Build history of the part. All positions in model axes, mm. A direction names the side the tool comes from. Round coordinates to 2 decimals unless told otherwise and drop trailing zeros. Write each loop counter-clockwise with the first axis right and the second up, starting at its lowest first coordinate (ties: lowest second). Pieces come first, ordered by that corner, then holes.
Item 1: Band-saw the part on A-A, the plane z = 50. Write the cut outline in (x, y), then the cut area to 3 significant figures.
Item 2: Band-saw the part on C-C, the plane y = 86.5. Write the cut outline in (x, z).
Item 3: Mould opens along Z. For faces 1 (the flat face through (-1, 51, 130)), 2 (the flat face through (-7, 42, -2)), 3 (the flat face through (-75, 46, -80)), 4 (the flat face through (-75, 46, 80)) say: +Z half, -Z half, draft (parallel to the pull), parting line (faces both ways), or undercut.
Item 4: Band-saw the part on D-D, the plane x = -76. Write the cut outline in (y, z).
Item 5: Wall check: probe 1 along Z at (x, y) = (60, 15); probe 2 along Z at (x, y) = (69.5, 25.5); probe 3 along X at (y, z) = (12, -50). Give the ranges that are in metal, low to high.
Item 6: 3-axis set-ups, long thin cutter, end or side, ignore diameter. For faces 5 (the cylindrical face through (30.007, 59.704, -50.66)), 6 (the flat face through (-71, 25, 50)), 7 (the flat face through (7, 42, -2)): which of +Z, -Z, +X, -X, +Y, -Y reach the whole face in a straight line?
Item 7: Drop flat-ended pins along their axis: pin 1 Ø1.5 at (x, z) = (-45.5, 25.5) entering from +Y; pin 2 Ø18.5 at (x, y) = (-87.5, 60.5) entering from -Z; pin 3 Ø2 at (x, z) = (-32, -18) entering from -Y; pin 4 Ø2 at (x, z) = (-16.5, -0.5) entering from +Y. Give the stop position or say it passes through.
Item 8: Band-saw the part on B-B, the plane z = 3. Write the cut outline in (x, y), then the cut area to 3 significant figures.
```python
from build123d import *

# Parameters (mm, degrees)
HOUSING_BODY_DEPTH                     = 130
BOLT_START                             = 25
BOLT_POCKET_DEPTH                      = 260
BOLT_POCKET_MIRROR_RIGHT_COPY_1_DEPTH  = 260
BOLT_HOLE_SKETCH_R                     = 10
BOLT_HOLE_20_DEPTH                     = 260
BOLT_HOLE_MIRROR_RIGHT_COPY_1_SKETCH_R = 10
BOLT_HOLE_MIRROR_RIGHT_COPY_1_DEPTH    = 260
NOTCH_CUT_DEPTH                        = 296.972971894


with BuildPart() as part:
    # Housing Profile Sketch → Housing Body (new, symmetric)
    with BuildSketch(Plane.XY):
        with BuildLine():
            Line((-100, 0), (-37.5, 0))
            ThreePointArc((-37.5, 0), (0, 37.5), (37.5, 0))
            Line((37.5, 0), (100, 0))
            ThreePointArc((100, 0), (0, 100), (-100, 0))
        make_face()
    extrude(amount=HOUSING_BODY_DEPTH, both=True)

    # Bolt Pocket Sketch → Bolt Pocket (cut)
    with BuildSketch(Plane(origin=(0, 0, 0), x_dir=(1, 0, 0), z_dir=(0, 1, 0)).offset(BOLT_START)):
        with BuildLine():
            Line((-60, -20), (-100, -20))
            Line((-100, -20), (-100, -80))
            Line((-100, -80), (-60, -80))
            ThreePointArc((-60, -80), (-30, -50), (-60, -20))
        make_face()
    bolt_pocket = extrude(amount=BOLT_POCKET_DEPTH, mode=Mode.SUBTRACT)

    # Bolt Pocket Mirror Front: Bolt Pocket across plane
    add(bolt_pocket.mirror(Plane.XY), mode=Mode.SUBTRACT)

    # Bolt Pocket Mirror Right: Bolt Pocket across plane
    add(bolt_pocket.mirror(Plane(origin=(0, 0, 0), x_dir=(0, 0, 1), z_dir=(1, 0, 0))), mode=Mode.SUBTRACT)

    # Bolt Pocket Mirror Right copy 1 sketch → Bolt Pocket Mirror Right copy 1 (cut)
    with BuildSketch(Plane(origin=(0, 0, 0), x_dir=(-1, 0, 0), z_dir=(0, 1, 0)).offset(BOLT_START)):
        with BuildLine():
            Line((-60, -20), (-100, -20))
            Line((-100, -20), (-100, -80))
            Line((-100, -80), (-60, -80))
            ThreePointArc((-60, -80), (-30, -50), (-60, -20))
        make_face()
    extrude(amount=BOLT_POCKET_MIRROR_RIGHT_COPY_1_DEPTH, mode=Mode.SUBTRACT)

    # Bolt Hole Sketch → Bolt Hole Ø20 (cut)
    with BuildSketch(Plane(origin=(0, 25, 0), x_dir=(1, 0, 0), z_dir=(0, 1, 0))):
        with Locations(Location((-60, -50, 0), (0, 0, 270))):
            Circle(BOLT_HOLE_SKETCH_R)
    bolt_hole_20 = extrude(amount=-BOLT_HOLE_20_DEPTH, mode=Mode.SUBTRACT)

    # Bolt Hole Mirror Front: Bolt Hole Ø20 across plane
    add(bolt_hole_20.mirror(Plane.XY), mode=Mode.SUBTRACT)

    # Bolt Hole Mirror Right: Bolt Hole Ø20 across plane
    add(bolt_hole_20.mirror(Plane(origin=(0, 0, 0), x_dir=(0, 0, 1), z_dir=(1, 0, 0))), mode=Mode.SUBTRACT)

    # Bolt Hole Mirror Right copy 1 sketch → Bolt Hole Mirror Right copy 1 (cut)
    with BuildSketch(Plane(origin=(0, 25, 0), x_dir=(-1, 0, 0), z_dir=(0, 1, 0))):
        with Locations(Location((-60, -50, 0), (0, 0, 270))):
            Circle(BOLT_HOLE_MIRROR_RIGHT_COPY_1_SKETCH_R)
    extrude(amount=-BOLT_HOLE_MIRROR_RIGHT_COPY_1_DEPTH, mode=Mode.SUBTRACT)

    # Notch Sketch → Notch Cut (cut, through all)
    with BuildSketch(Plane(origin=(0, 0, -130), x_dir=(-1, 0, 0), z_dir=(0, 0, -1))):
        with BuildLine():
            Line((-7, 47.84087404), (7, 47.84087404))
            Line((7, 47.84087404), (7, 36.84087404))
            ThreePointArc((7, 36.84087404), (0, 37.5), (-7, 36.84087404))
            Line((-7, 36.84087404), (-7, 47.84087404))
        make_face()
    extrude(amount=-NOTCH_CUT_DEPTH, mode=Mode.SUBTRACT)


solid = part.part
```
Results:
1. outline: (-100, 0) - (-70, 0) - (-70, 25) - (-96.82, 25) arc R100 ccw to start; (-50, 0) - (-37.5, 0) arc R37.5 cw to (-7, 36.84) - (-7, 47.84) - (7, 47.84) - (7, 36.84) arc R37.5 cw to (37.5, 0) - (50, 0) - (50, 25) - (30, 25) - (30, 95.39) arc R100 ccw to (-30, 95.39) - (-30, 25) - (-50, 25) - close; (70, 0) - (100, 0) arc R100 ccw to (96.82, 25) - (70, 25) - close
1. area: 6,000 mm2
2. outline: (-50.18, -130) - (50.18, -130) - (50.18, -78.35) arc R30 cw to (50.18, -21.65) - (50.18, 21.65) arc R30 cw to (50.18, 78.35) - (50.18, 130) - (-50.18, 130) - (-50.18, 78.35) arc R30 cw to (-50.18, 21.65) - (-50.18, -21.65) arc R30 cw to (-50.18, -78.35) - close
3. face 1: +Z half
3. face 2: draft
3. face 3: undercut
3. face 4: undercut
4. outline: (0, -130) - (64.99, -130) - (64.99, -80) - (25, -80) - (25, -20) - (64.99, -20) - (64.99, 20) - (25, 20) - (25, 80) - (64.99, 80) - (64.99, 130) - (0, 130) - close
5. probe 1: z = -130 to -60, -40 to 40, 60 to 130
5. probe 2: z = -130 to -80, -20 to 20, 80 to 130
5. probe 3: x = -99.28 to -70, -50 to -35.53, 35.53 to 50, 70 to 99.28
6. face 5: +X, +Y
6. face 6: -X, +Y
6. face 7: +Z, -Z, -Y
7. pin 1: stops at y = 25
7. pin 2: stops at z = -130
7. pin 3: stops at y = 17.81
7. pin 4: stops at y = 98.79
8. outline: (-100, 0) - (-37.5, 0) arc R37.5 cw to (-7, 36.84) - (-7, 47.84) - (7, 47.84) - (7, 36.84) arc R37.5 cw to (37.5, 0) - (100, 0) arc R100 ccw to start
8. area: 13,400 mm2
